Here's how the part is built. I have some questions about the finished solid (model axes, mm). A direction names the side the tool comes from. Coordinates: 2 decimals unless noted, no trailing zeros. Loops run counter-clockwise (first coordinate to the right, second up) from the corner with the lowest first, then second, coordinate; pieces in that order, holes last. Notation, with made-up numbers: (60, -16.5) -> (108, -16.5) arc R30 ccw to (108, 15.5) -> close; hole circle Ø1 at (-21.5, 83). An arc over 180 degrees is marked (long way). Answer as a JSON object with one key per item and string values. Group by question number.
1) I need wall thicknesses on probe 1 along Y at (x, z) = (29, -146); probe 2 along X at (y, z) = (8, -187); probe 3 along Z at (x, y) = (68.5, 17). Which ranges of each line are inside material? Lowest first, please. Write a range as [from, to].
2) I'm going to push flat-ended pins straight in: pin 1 (17 mm diameter, centred on y = 96, z = -70, fed in from +X); pin 2 (1 mm diameter, centred on x = 27, z = -32, fed in from -Y); pin 3 (7 mm diameter, centred on x = 26.5, y = -5, fed in from +Z). Where does each tip first touch, or does it pass through?
3) I want a section at B-B (y = 96). Write out the boundary of the cut face in (x, z), then the cut area to 3 significant figures.
4) If we mould it in two halves opening along Y, with no side actions, what happens to faces 1 (the flat face through (47, 39, -118)), 2 (the flat face through (50, -9, -107)), 3 (the cylindrical face through (29.86, 112.021, -156.214))? For each: +Y half, -Y half, draft (parallel to the pull), parting line (faces both ways), or undercut.
5) I want a section at A-A (z = -146). Write out the boundary of the cut face in (x, y).
6) I want a section at C-C (x = 47). Write out the boundary of the cut face in (y, z).
7) Which directions (+Z, -Z, +X, -X, +Y, -Y) give clear straight access to the entire face, cutting with the end or side of a thin tool? Please do faces 4 (the flat face through (20, 73, -106)), 5 (the flat face through (50, 0, -28)), 6 (the flat face through (40, 92, -61)), 7 (the flat face through (50, 0, -187)).
8) I want a section at D-D (z = -187.5). Write out the boundary of the cut face in (x, y), then the cut area to 3 significant figures.
```python
from build123d import *

# Parameters (mm, degrees)
BASE_PLATE_DEPTH                = 102
UPRIGHT_PLATE_DEPTH             = 20
UPRIGHT_BOSS_1_PROFILE_R        = 19
UPRIGHT_BOSS_1_PROFILE_R_2      = 9.5
UPRIGHT_BOSS_1_DEPTH            = 20
UPRIGHT_BOSS_2_PROFILE_R        = 19
UPRIGHT_BOSS_2_PROFILE_R_2      = 9.5
UPRIGHT_BOSS_2_DEPTH            = 20
BASE_POCKET_1_PROFILE_R         = 19
BASE_POCKET_1_DEPTH             = 9
MOUNTING_HOLE_1_PROFILE_R       = 9.5
MOUNTING_HOLE_1_DEPTH           = 265.680940001
BASE_POCKET_2_PROFILE_R         = 19
BASE_POCKET_2_DEPTH             = 9
MOUNTING_HOLE_2_PROFILE_R       = 9.5
MOUNTING_HOLE_2_DEPTH           = 265.680940001
UPRIGHT_CORNER_FILLET_R26_1_R   = 26
UPRIGHT_CORNER_FILLET_R26_2_R   = 26
BASE_CORNER_FILLETS_R26_R       = 26
GUSSET_RIB_REACH                = 196.147
GUSSET_RIB_PROFILE_30DEG_WALL_W = 484.979147418
GUSSET_RIB_PROFILE_30DEG_WALL_H = 20


with BuildPart() as part:
    # Base Plate Profile → Base Plate (new body)
    with BuildSketch(Plane(origin=(0, 0, 0), x_dir=(0, 0, -1), z_dir=(1, 0, 0))):
        Polygon((0, 0), (57, 0), (57, -9), (159, -9), (159, 0), (216, 0), (216, 20), (0, 20), align=None)
    extrude(amount=BASE_PLATE_DEPTH)

    # Upright Plate Profile → Upright Plate (add)
    with BuildSketch(Plane(origin=(0, 0, 0), x_dir=(0, 0, -1), z_dir=(1, 0, 0))):
        Polygon((0, 20), (216, 20), (172, 125), (44, 125), align=None)
    extrude(amount=UPRIGHT_PLATE_DEPTH)

    # Upright Boss 1 Profile → Upright Boss 1 (add)
    with BuildSketch(Plane(origin=(20, 0, 0), x_dir=(0, 0, -1), z_dir=(1, 0, 0))):
        with Locations((70, 96)):
            Circle(UPRIGHT_BOSS_1_PROFILE_R)
        with Locations((70, 96)):
            Circle(UPRIGHT_BOSS_1_PROFILE_R_2, mode=Mode.SUBTRACT)
    extrude(amount=UPRIGHT_BOSS_1_DEPTH)

    # Upright Boss 2 Profile → Upright Boss 2 (add)
    with BuildSketch(Plane(origin=(20, 0, 0), x_dir=(0, 0, -1), z_dir=(1, 0, 0))):
        with Locations((146, 96)):
            Circle(UPRIGHT_BOSS_2_PROFILE_R)
        with Locations((146, 96)):
            Circle(UPRIGHT_BOSS_2_PROFILE_R_2, mode=Mode.SUBTRACT)
    extrude(amount=UPRIGHT_BOSS_2_DEPTH)

    # Base Pocket 1 Profile → Base Pocket 1 (cut)
    with BuildSketch(Plane(origin=(0, 20, 0), x_dir=(1, 0, 0), z_dir=(0, 1, 0))):
        with Locations(Location((73, 187.5, 0), (0, 0, 270))):
            Circle(BASE_POCKET_1_PROFILE_R)
    extrude(amount=-BASE_POCKET_1_DEPTH, mode=Mode.SUBTRACT)

    # Mounting Hole 1 Profile → Mounting Hole 1 (cut, through all)
    with BuildSketch(Plane(origin=(0, 11, 0), x_dir=(1, 0, 0), z_dir=(0, 1, 0))):
        with Locations(Location((73, 187.5, 0), (0, 0, 270))):
            Circle(MOUNTING_HOLE_1_PROFILE_R)
    extrude(amount=-MOUNTING_HOLE_1_DEPTH, mode=Mode.SUBTRACT)

    # Base Pocket 2 Profile → Base Pocket 2 (cut)
    with BuildSketch(Plane(origin=(0, 20, 0), x_dir=(1, 0, 0), z_dir=(0, 1, 0))):
        with Locations(Location((70.69, 28.5, 0), (0, 0, 270))):
            Circle(BASE_POCKET_2_PROFILE_R)
    extrude(amount=-BASE_POCKET_2_DEPTH, mode=Mode.SUBTRACT)

    # Mounting Hole 2 Profile → Mounting Hole 2 (cut, through all)
    with BuildSketch(Plane(origin=(0, 11, 0), x_dir=(1, 0, 0), z_dir=(0, 1, 0))):
        with Locations(Location((70.69, 28.5, 0), (0, 0, 270))):
            Circle(MOUNTING_HOLE_2_PROFILE_R)
    extrude(amount=-MOUNTING_HOLE_2_DEPTH, mode=Mode.SUBTRACT)

    # Upright Corner Fillet R26 1
    upright_corner_fillet_r26_1_edges = [part.edges().sort_by_distance(p)[0] for p in [
        (10, 125, -44),
    ]]
    fillet(upright_corner_fillet_r26_1_edges, radius=UPRIGHT_CORNER_FILLET_R26_1_R)

    # Upright Corner Fillet R26 2
    upright_corner_fillet_r26_2_edges = [part.edges().sort_by_distance(p)[0] for p in [
        (10, 125, -172),
    ]]
    fillet(upright_corner_fillet_r26_2_edges, radius=UPRIGHT_CORNER_FILLET_R26_2_R)

    # Base Corner Fillets R26
    base_corner_fillets_r26_edges = [part.edges().sort_by_distance(p)[0] for p in [
        (102, 10, -216),
        (102, 10, 0),
    ]]
    fillet(base_corner_fillets_r26_edges, radius=BASE_CORNER_FILLETS_R26_R)

    # Gusset Rib Profile 30deg wall → Gusset Rib (add, up to next)
    with BuildSketch(Plane(origin=(61, 43.671361037, -108), x_dir=(-0.866025403782, 0.500000000004, 0), z_dir=(-0.500000000004, -0.866025403782, 0)), mode=Mode.PRIVATE) as gusset_rib_sk1:
        Rectangle(GUSSET_RIB_PROFILE_30DEG_WALL_W, GUSSET_RIB_PROFILE_30DEG_WALL_H)
    gusset_rib_tool1 = extrude(gusset_rib_sk1.sketch, amount=GUSSET_RIB_REACH, mode=Mode.PRIVATE) - part.part
    add(gusset_rib_tool1.solids().sort_by_distance((61, 43.671361037, -108))[0])


solid = part.part
```
Determined:
{
 "1": {"probe 1": "[-9, 20], [77, 86.5], [105.5, 115]", "probe 2": "[0, 63.51], [82.49, 102]", "probe 3": "[-216, -205.96], [-169.04, -47.37], [-9.63, 0]"},
 "2": {"pin 1": "x = 20", "pin 2": "y = 0", "pin 3": "z = -57"},
 "3": {"outline": "(0, -184.15) -> (20, -184.15) -> (20, -165) -> (40, -165) -> (40, -155.5) -> (20, -155.5) -> (20, -136.5) -> (40, -136.5) -> (40, -127) -> (20, -127) -> (20, -89) -> (40, -89) -> (40, -79.5) -> (20, -79.5) -> (20, -60.5) -> (40, -60.5) -> (40, -51) -> (20, -51) -> (20, -31.85) -> (0, -31.85) -> close", "area": "3,810 mm^2"},
 "4": {"face 1": "draft", "face 2": "-Y half", "face 3": "undercut"},
 "5": {"outline": "(0, -9) -> (102, -9) -> (102, 20) -> (20, 20) -> (20, 77) -> (40, 77) -> (40, 86.5) -> (20, 86.5) -> (20, 105.5) -> (40, 105.5) -> (40, 115) -> (20, 115) -> (20, 125) -> (0, 125) -> close"},
 "6": {"outline": "(-9, -159) -> (0, -159) -> (0, -216) -> (20, -216) -> (20, -118) -> (51.75, -118) -> (51.75, -98) -> (20, -98) -> (20, 0) -> (0, 0) -> (0, -57) -> (-9, -57) -> close"},
 "7": {"face 4": "+X", "face 5": "+Z, +X, -X, -Y", "face 6": "+Z, -Z, +X, +Y", "face 7": "-Z, +X, -X, -Y"},
 "8": {"outline": "(0, 0) -> (63.5, 0) -> (63.5, 11) -> (54, 11) -> (54, 20) -> (20, 20) -> (20, 88.01) -> (0, 88.01) -> close; (82.5, 0) -> (102, 0) -> (102, 20) -> (92, 20) -> (92, 11) -> (82.5, 11) -> close", "area": "2,850 mm^2"}
}
